from build123d import *

# Parameters (mm, degrees)
SKETCH1_W                  = 40
SKETCH1_H                  = 80
BOSS_EXTRUDE1_DEPTH        = 10
F_11_0_11_DIAMETER_HOLE1_D = 11


with BuildPart() as part:
    # Sketch1 → Boss-Extrude1 (new body)
    with BuildSketch(Plane.XY):
        with Locations((20, 40)):
            Rectangle(SKETCH1_W, SKETCH1_H)
    extrude(amount=BOSS_EXTRUDE1_DEPTH)

    # Ø11.0 (11) Diameter Hole1 (through all)
    with Locations(Plane.XY.offset(10)):
        with Locations((20, 40)):
            Hole(F_11_0_11_DIAMETER_HOLE1_D / 2)


solid = part.part
Input: part model. Units: mm. Frame: model coordinates. Give positions to 0.01 mm unless a question says otherwise; leave off trailing zeros. Write each loop counter-clockwise with the first axis right and the second up, starting at its lowest first coordinate (ties: lowest second). Pieces come first, ordered by that corner, then holes.
Q1. Material intervals for probe 1 along Y at (x, z) = (20, 7.5); probe 2 along Y at (x, z) = (16, 5.75), sorted ascending.
Q2. Section A-A, the plane x = 20. Output: boundary loops of the cut face in (y, z), plus the area to 3 significant figures.
Q3. Section B-B, the plane z = 7.75. Output: boundary loops of the cut face in (x, y), plus the area to 3 significant figures.
Q4. Pull-direction query (Y, two-part tool) for faces 1 (the face through (20.716, 45.453, 4.93)), 2 (the face through (0, 39, 5)), 3 (the face through (20, 80, 5)); classes: pulls with the +Y half, pulls with the -Y half, needs draft (parallel to the pull), parting line crosses it, or undercut.
Filled in:
1. probe 1: y = 0 to 34.5, 45.5 to 80
1. probe 2: y = 0 to 36.23, 43.77 to 80
2. outline: (0, 0) - (34.5, 0) - (34.5, 10) - (0, 10) - close; (45.5, 0) - (80, 0) - (80, 10) - (45.5, 10) - close
2. area: 690 mm2
3. outline: (0, 0) - (40, 0) - (40, 80) - (0, 80) - close; hole circle Ø11 at (20, 40)
3. area: 3,100 mm2
4. face 1: undercut
4. face 2: needs draft
4. face 3: pulls with the +Y half
